from build123d import *

# Parameters (mm, degrees)
SKETCH1_R           = 2.5
BOSS_EXTRUDE1_DEPTH = 10.5
SKETCH2_R           = 3
BOSS_EXTRUDE2_DEPTH = 1
BOSS_EXTRUDE3_START = 1
SKETCH3_R           = 3
BOSS_EXTRUDE3_DEPTH = 1
DOME1_FACE_RADIUS   = 3
DOME1_HEIGHT        = 0.5
DOME2_FACE_RADIUS   = 3
DOME2_HEIGHT        = 0.5


with BuildPart() as part:
    # Sketch1 → Boss-Extrude1 (new, symmetric)
    with BuildSketch(Plane.XY):
        with Locations(Location((0, 0, 0), (0, 0, 180))):
            Circle(SKETCH1_R)
    extrude(amount=BOSS_EXTRUDE1_DEPTH, both=True)

    # Sketch2 → Boss-Extrude2 (add)
    with BuildSketch(Plane(origin=(0, 0, -10.5), x_dir=(-1, 0, 0), z_dir=(0, 0, -1))):
        Circle(SKETCH2_R)
    extrude(amount=BOSS_EXTRUDE2_DEPTH)

    # Sketch3 → Boss-Extrude3 (add)
    with BuildSketch(Plane.XY.offset(10.5).offset(BOSS_EXTRUDE3_START)):
        with Locations(Location((0, 0, 0), (0, 0, 180))):
            Circle(SKETCH3_R)
    extrude(amount=-BOSS_EXTRUDE3_DEPTH)

    # Dome1: a dome of height H over a round flat face of radius A is a cap of a sphere of radius (A * A + H * H) / (2 * H)
    dome1_r = (DOME1_FACE_RADIUS * DOME1_FACE_RADIUS + DOME1_HEIGHT * DOME1_HEIGHT) / (2 * DOME1_HEIGHT)
    dome1_base = Plane((0, 0, -11.5), z_dir=(0, 0, -1))
    with Locations(dome1_base.offset(DOME1_HEIGHT - dome1_r)):
        dome1_ball = Sphere(dome1_r, mode=Mode.PRIVATE)
    add(split(dome1_ball, bisect_by=dome1_base, keep=Keep.TOP, mode=Mode.PRIVATE))

    # Dome2: a dome of height H over a round flat face of radius A is a cap of a sphere of radius (A * A + H * H) / (2 * H)
    dome2_r = (DOME2_FACE_RADIUS * DOME2_FACE_RADIUS + DOME2_HEIGHT * DOME2_HEIGHT) / (2 * DOME2_HEIGHT)
    dome2_base = Plane((0, 0, 11.5), z_dir=(0, 0, 1))
    with Locations(dome2_base.offset(DOME2_HEIGHT - dome2_r)):
        dome2_ball = Sphere(dome2_r, mode=Mode.PRIVATE)
    add(split(dome2_ball, bisect_by=dome2_base, keep=Keep.TOP, mode=Mode.PRIVATE))


solid = part.part
Here's how the part is built. I have some questions about the finished solid (model axes, mm). A direction names the side the tool comes from. Round coordinates to 2 decimals unless told otherwise and drop trailing zeros. Write each loop counter-clockwise with the first axis right and the second up, starting at its lowest first coordinate (ties: lowest second). Pieces come first, ordered by that corner, then holes. Notation, with made-up numbers: (-14.5, -1) -> (34.5, -1) arc R25 ccw to (34.5, 11) -> close; hole circle Ø2 at (71.5, 14.25). An arc over 180 degrees is marked (long way). One line per item, written item: value.
1) Suppose I cut it at C-C on z = 2.75. List the corners of the cut face in (x, y) for me.
Filled sheet:
outline: circle Ø5 at (0, 0)
2) Suppose I cut it at B-B on y = 0. List the corners of the cut face in (x, z) for me.
Filled sheet:
outline: (-3, -11.5) arc R9.25 ccw to (3, -11.5) -> (3, -10.5) -> (2.5, -10.5) -> (2.5, 10.5) -> (3, 10.5) -> (3, 11.5) arc R9.25 ccw to (-3, 11.5) -> (-3, 10.5) -> (-2.5, 10.5) -> (-2.5, -10.5) -> (-3, -10.5) -> close
3) If I drill on line 1 (Z direction, x = 2, y = -1.6); line 2 (Z direction, x = 2, y = 2.15); line 3 (Z direction, x = 0, y = 2.25), over which ranges is the centre line in solid material (lowest first)? Write a range as [from, to].
Filled sheet:
line 1: z = [-11.64, -10.5], [10.5, 11.64]
line 2: z = [-11.52, -10.5], [10.5, 11.52]
line 3: z = [-11.72, 11.72]
4) Suppose I cut it at A-A on x = -0.25. List the corners of the cut face in (y, z) for me.
Filled sheet:
outline: (-2.99, -11.5) arc R9.25 ccw to (2.99, -11.5) -> (2.99, -10.5) -> (2.49, -10.5) -> (2.49, 10.5) -> (2.99, 10.5) -> (2.99, 11.5) arc R9.25 ccw to (-2.99, 11.5) -> (-2.99, 10.5) -> (-2.49, 10.5) -> (-2.49, -10.5) -> (-2.99, -10.5) -> close
5) For faces 3 (the face through (2, 2, -10.5)), 4 (the face through (-2.86, -0.9, 11.01)), which set-ups out of +Z, -Z, +X, -X, +Y, -Y let a thin tool reach every point of the face, with its end or its side?
Filled sheet:
face 3: none
face 4: +Z, -Z
6) I'm going to push flat-ended pins straight in: pin 1 Ø1.5 at (y, z) = (0.5, 9) entering from +X; pin 2 Ø3 at (x, z) = (2, 3.5) entering from +Y; pin 3 Ø3 at (x, y) = (1.5, 1) entering from -Z. Where does each tip first touch, or does it pass through?
Filled sheet:
pin 1: stops at x = 2.5
pin 2: stops at y = 2.45
pin 3: stops at z = -12
7) We'd pull the mould along Z, two halves only. Please class faces 1 (the face through (3, 0, -11)), 2 (the face through (2, -2, 10.5)): released by +Z, released by -Z, zero draft, split by the parting line, or undercut.
Filled sheet:
face 1: zero draft
face 2: undercut
